Model file for the job. Use its own axes, mm. A direction names the side the tool comes from. Coordinates: 2 decimals unless noted, no trailing zeros. Loops run counter-clockwise (first coordinate to the right, second up) from the corner with the lowest first, then second, coordinate; pieces in that order, holes last.
from build123d import *

# Parameters (mm, degrees)
SKETCH_1_W             = 126
SKETCH_1_H             = 10
EXTRUDE_1_DEPTH        = 43.6
CHAMFER_1_SIZE         = 5
HOLE_WIZARD_M4_1_D     = 3.3
HOLE_WIZARD_M4_1_DEPTH = 10.1
HOLE_WIZARD_M4_1_TIP   = 0.991420021
HOLE_WIZARD_M5_1_D     = 4.2


with BuildPart() as part:
    # 草图1 → 凸台-拉伸1 (new body)
    with BuildSketch(Plane(origin=(0, 0, 0), x_dir=(1, 0, 0), z_dir=(0, 1, 0))):
        with Locations((63, 5)):
            Rectangle(SKETCH_1_W, SKETCH_1_H)
    extrude(amount=EXTRUDE_1_DEPTH)

    # 倒角1
    chamfer_1_edges = [part.edges().sort_by_distance(p)[0] for p in [
        (126, 43.6, -5),
        (126, 0, -5),
    ]]
    chamfer(chamfer_1_edges, length=CHAMFER_1_SIZE)

    # M4 螺纹孔1
    with Locations(Plane.ZY):
        with Locations((-5, 36.8), (-5, 21.783451384), (-5, 6.8)):
            Hole(HOLE_WIZARD_M4_1_D / 2, depth=HOLE_WIZARD_M4_1_DEPTH)
            with Locations((0, 0, -(HOLE_WIZARD_M4_1_DEPTH + HOLE_WIZARD_M4_1_TIP / 2))):  # 118° drill point
                Cone(0, HOLE_WIZARD_M4_1_D / 2, HOLE_WIZARD_M4_1_TIP, mode=Mode.SUBTRACT)

    # M5 螺纹孔1 (through all)
    with Locations(Plane(origin=(0, 0, -10), x_dir=(-1, 0, 0), z_dir=(0, 0, -1))):
        with Locations((-40.5, 33.55), (-40.5, 10.05), (-118.5, 33.55), (-118.5, 10.05)):
            Hole(HOLE_WIZARD_M5_1_D / 2)


solid = part.part
Q1. Drill centre lines: line 1 (Y direction, x = 40.5, z = -6.5); line 2 (X direction, y = 11, z = -3.25); line 3 (Z direction, x = 6.25, y = 6.8). Where is each one in solid material? Low to high.
Answers:
line 1: y = 0 to 7.95, 12.15 to 31.45, 35.65 to 43.6
line 2: x = 0 to 38.63, 42.37 to 116.63, 120.37 to 126
line 3: z = -10 to -6.65, -3.35 to 0
Q2. Slice it at B-B (x = 40.5). List the corners of the cut face in (y, z).
Answers:
outline: (0, -10) - (7.95, -10) - (7.95, 0) - (0, 0) - close; (12.15, -10) - (31.45, -10) - (31.45, 0) - (12.15, 0) - close; (35.65, -10) - (43.6, -10) - (43.6, 0) - (35.65, 0) - close
Q3. Mould opens along Z. For faces 1 (the flat face through (62, 21, -10)), 2 (the conical face through (10.92, 37.08, -5.04)), 3 (the cylindrical face through (120.44, 9.25, -4.93)) say: +Z half, -Z half, draft (parallel to the pull), parting line (faces both ways), or undercut.
Answers:
face 1: -Z half
face 2: undercut
face 3: draft
Q4. Slice it at A-A (y = 33.55). List the corners of the cut face in (x, z).
Answers:
outline: (0, -10) - (38.4, -10) - (38.4, 0) - (0, 0) - close; (42.6, -10) - (116.4, -10) - (116.4, 0) - (42.6, 0) - close; (120.6, -10) - (126, -10) - (126, 0) - (120.6, 0) - close
Q5. Which spindle directions (+Z, -Z, +X, -X, +Y, -Y) get a long thin tool onto all of the face, cutting with end or side? Do faces 4 (the cylindrical face through (119.63, 35.32, -4.93)), 5 (the cylindrical face through (5.121, 20.173, -4.642)). Say none if no direction does.
Answers:
face 4: +Z, -Z
face 5: -X
